Build history of the part. All positions in model axes, mm. A direction names the side the tool comes from. Give positions to 0.01 mm unless a question says otherwise; leave off trailing zeros. Write each loop counter-clockwise with the first axis right and the second up, starting at its lowest first coordinate (ties: lowest second). Pieces come first, ordered by that corner, then holes.
from build123d import *

# Parameters (mm, degrees)
SKETCH_1_R                   = 7.5
EXTRUDE_1_DEPTH              = 207
SKETCH_2_R                   = 10
EXTRUDE_2_DEPTH              = 68
SKETCH_3_OUTSIDE_W           = 77.29
SKETCH_3_OUTSIDE_H           = 77.29
SKETCH_3_OUTSIDE_W_2         = 23
SKETCH_3_OUTSIDE_H_2         = 18
CUT_EXTRUDE_1_DEPTH          = 20
HOLE_WIZARD_M8_1_D           = 6.8
HOLE_WIZARD_M8_1_DEPTH       = 18.25
HOLE_WIZARD_M8_1_CSINK_D     = 8.05
HOLE_WIZARD_M8_1_CSINK_ANGLE = 90
HOLE_WIZARD_M8_1_TIP         = 2.042926105


with BuildPart() as part:
    # 草图1 → 凸台-拉伸1 (new body)
    with BuildSketch(Plane.XY):
        Circle(SKETCH_1_R)
    extrude(amount=EXTRUDE_1_DEPTH)

    # 草图2 → 凸台-拉伸2 (add)
    with BuildSketch(Plane(origin=(0, 0, 0), x_dir=(-1, 0, 0), z_dir=(0, 0, -1))):
        Circle(SKETCH_2_R)
    extrude(amount=EXTRUDE_2_DEPTH)

    # 草图3 outside → 切除-拉伸1 (cut)
    with BuildSketch(Plane(origin=(0, 0, -68), x_dir=(-1, 0, 0), z_dir=(0, 0, -1))):
        Rectangle(SKETCH_3_OUTSIDE_W, SKETCH_3_OUTSIDE_H)
        Rectangle(SKETCH_3_OUTSIDE_W_2, SKETCH_3_OUTSIDE_H_2, mode=Mode.SUBTRACT)
    extrude(amount=-CUT_EXTRUDE_1_DEPTH, mode=Mode.SUBTRACT)

    # M8 螺纹孔1
    with Locations(Plane(origin=(0, 0, -68), x_dir=(-1, 0, 0), z_dir=(0, 0, -1))):
        with Locations((0, 0)):
            CounterSinkHole(HOLE_WIZARD_M8_1_D / 2, HOLE_WIZARD_M8_1_CSINK_D / 2, depth=HOLE_WIZARD_M8_1_DEPTH, counter_sink_angle=HOLE_WIZARD_M8_1_CSINK_ANGLE)
            with Locations((0, 0, -(HOLE_WIZARD_M8_1_DEPTH + HOLE_WIZARD_M8_1_TIP / 2))):  # 118° drill point
                Cone(0, HOLE_WIZARD_M8_1_D / 2, HOLE_WIZARD_M8_1_TIP, mode=Mode.SUBTRACT)


solid = part.part
1. Drop flat-ended pins along their axis: pin 1 (8 mm diameter, centred on y = 4, z = 100.5, fed in from +X); pin 2 (6 mm diameter, centred on x = -1.5, z = 33, fed in from -Y); pin 3 (2.5 mm diameter, centred on x = 1.5, z = -56, fed in from -Y). Give the stop position or say it passes through.
2. Saw through at A-A on z = 137. Give the cut face in (x, y), plus the area to 3 significant figures.
3. Drill centre lines: line 1 along Y through (x, z) = (0, -57.75); line 2 along X through (y, z) = (0, -60.5); line 3 along Z through (x, y) = (8.25, 4). Where is each one in solid material? Low to high.
4. Mould opens along Y. For faces 1 (the face through (0, 9, -58)), 2 (the face through (-0.74, -3.32, -58.44)), 3 (the face through (-4.3, 0.1, -68)) say: pulls with the +Y half, pulls with the -Y half, needs draft (parallel to the pull), parting line crosses it, or undercut.
5. 3-axis set-ups, long thin cutter, end or side, ignore diameter. For faces 4 (the face through (0.128, -0.576, -48.062)), 5 (the face through (0, -9, -58)), 6 (the face through (-7.493, 0.33, 102.051)): which of +Z, -Z, +X, -X, +Y, -Y reach the whole face in a straight line?
Outcome:
1. pin 1: stops at x = 7.5
1. pin 2: stops at y = -7.5
1. pin 3: stops at y = -9
2. outline: circle Ø15 at (0, 0)
2. area: 177 mm2
3. line 1: y = -9 to -3.4, 3.4 to 9
3. line 2: x = -10 to -3.4, 3.4 to 10
3. line 3: z = -68 to 0
4. face 1: pulls with the +Y half
4. face 2: undercut
4. face 3: needs draft
5. face 4: -Z
5. face 5: -Z, +X, -X, -Y
5. face 6: +Z
